Source: CAD feature listing. Evaluate the final solid. Frame: model axes, mm. Face numbers are marked on the shaded views. A direction names the side the tool comes from. Round coordinates to 2 decimals unless told otherwise and drop trailing zeros. Loops run counter-clockwise (first coordinate to the right, second up) from the corner with the lowest first, then second, coordinate; pieces in that order, holes last.
Item 1: Section query D-D on x = 3.5. Return loops of the section in (y, z), then the cut area to 3 significant figures.
Item 2: First-contact query: P1, Ø1, axis at x = 0.5, y = 2.5, coming from the +Z side. Flat tip, straight axial feed; report the tip coordinate or a pass-through.
Item 3: Ray query, L1, parallel to Z at x = 0, y = 2.5; L2, parallel to Y at x = 0, z = -2; L3, parallel to X at y = 0.5, z = 0.75. Return the intervals inside material, ascending.
Item 4: Pull-direction query (Y, two-part tool) for the marked faces 3 and 4; classes: released by +Y, released by -Y, zero draft, split by the parting line, or undercut.
Item 5: Section query C-C on z = 0.5. Return loops of the section in (x, y), then the cut area to 3 significant figures.
Item 6: Access query for the marked faces 1 and 2. Directions: +Z, -Z, +X, -X, +Y, -Y. A direction counts if a zero-diameter tool reaches every point of the face in a straight line with its end or side. Return the directions, or none.
Item 7: Section query A-A on x = 0. Return loops of the section in (y, z), then the cut area to 3 significant figures.
```python
from build123d import *

# Parameters (mm, degrees)
SKETCH_1_R           = 1.5
BOSS_EXTRUDE_1_DEPTH = 1
SKETCH_2_R           = 4
BOSS_EXTRUDE_2_DEPTH = 1
SKETCH_3_R           = 2.5
BOSS_EXTRUDE_3_DEPTH = 1
BOSS_EXTRUDE_START   = 4
SKETCH_4_R           = 1.5
BOSS_EXTRUDE_4_DEPTH = 4


with BuildPart() as part:
    # Sketch 1 → Boss-Extrude 1 (new body)
    with BuildSketch(Plane.XY):
        Circle(SKETCH_1_R)
    extrude(amount=BOSS_EXTRUDE_1_DEPTH)

    # Sketch 2 → Boss-Extrude 2 (add)
    with BuildSketch(Plane(origin=(0, 0, 0), x_dir=(-1, 0, 0), z_dir=(0, 0, -1))):
        Circle(SKETCH_2_R)
    extrude(amount=BOSS_EXTRUDE_2_DEPTH)

    # Sketch 3 → Boss-Extrude 3 (add)
    with BuildSketch(Plane(origin=(0, 0, -1), x_dir=(-1, 0, 0), z_dir=(0, 0, -1))):
        Circle(SKETCH_3_R)
    extrude(amount=BOSS_EXTRUDE_3_DEPTH)

    # Sketch 4 → Boss-Extrude 4 (add)
    with BuildSketch(Plane(origin=(0, 0, -2), x_dir=(-1, 0, 0), z_dir=(0, 0, -1)).offset(BOSS_EXTRUDE_START)):
        with Locations(Location((0, 0, 0), (0, 0, 180))):
            Circle(SKETCH_4_R)
    extrude(amount=-BOSS_EXTRUDE_4_DEPTH)

    # Sketch 5 → Cut-Revolve 2 (revolve, cut)
    with BuildSketch(Plane(origin=(0, 0, 0), x_dir=(1, 0, 0), z_dir=(0, 1, 0))):
        with BuildLine():
            Line((1.5, 2.003149648), (2.5, 2.000004945))
            Line((2.5, 2.000004945), (2.5, 1))
            ThreePointArc((2.5, 1), (1.791778774, 1.294007363), (1.5, 2.003149648))
        make_face()
    revolve(axis=Axis((0, 0, -2.003149648), (0, 0, -1)), mode=Mode.SUBTRACT)


solid = part.part
```
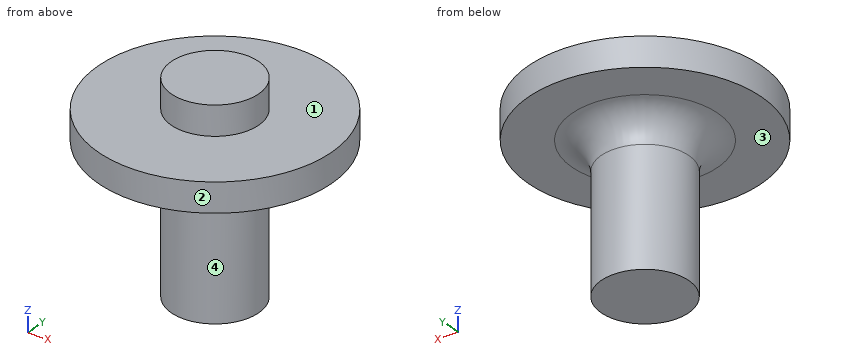
Data:
1. outline: (-1.94, -1) - (1.94, -1) - (1.94, 0) - (-1.94, 0) - close
1. area: 3.87 mm2
2. P1: stops at z = 0
3. L1: z = -1 to 0
3. L2: y = -1.5 to 1.5
3. L3: x = -1.41 to 1.41
4. face 3: zero draft
4. face 4: split by the parting line
5. outline: circle Ø3 at (0, 0)
5. area: 7.07 mm2
6. face 1: +Z
6. face 2: +Z, -Z
7. outline: (-4, -1) - (-2.5, -1) arc R1 cw to (-1.5, -2) - (-1.5, -6) - (1.5, -6) - (1.5, -2) arc R1 cw to (2.5, -1) - (4, -1) - (4, 0) - (1.5, 0) - (1.5, 1) - (-1.5, 1) - (-1.5, 0) - (-4, 0) - close
7. area: 26.4 mm2
